Part model, mm, in its own coordinate system. A direction names the side the tool comes from. Coordinates: 2 decimals unless noted, no trailing zeros. Loops run counter-clockwise (first coordinate to the right, second up) from the corner with the lowest first, then second, coordinate; pieces in that order, holes last. Notation, with made-up numbers: (-17, -36) - (-8, -36) arc R27 ccw to (-8, -16) - close; hole circle Ø7 at (9, -15). An arc over 180 degrees is marked (long way). Answer as CSV lines item,"result".
from build123d import *

# Parameters (mm, degrees)
BOSS_EXTRUDE1_DEPTH = 6.4
SKETCH3_R           = 5
BOSS_EXTRUDE2_DEPTH = 30
CHAMFER1_SIZE       = 1


with BuildPart() as part:
    # Sketch1 → Boss-Extrude1 (new body)
    with BuildSketch(Plane.XY):
        Polygon((8, 4.618802154), (0, 9.237604307), (-8, 4.618802154), (-8, -4.618802154), (0, -9.237604307), (8, -4.618802154), align=None)
    extrude(amount=BOSS_EXTRUDE1_DEPTH)

    # Sketch3 → Boss-Extrude2 (add)
    with BuildSketch(Plane.XY.offset(6.4)):
        Circle(SKETCH3_R)
    extrude(amount=BOSS_EXTRUDE2_DEPTH)

    # Chamfer1
    chamfer1_edges = [part.edges().sort_by_distance(p)[0] for p in [
        (-5, 0, 36.4),
    ]]
    chamfer(chamfer1_edges, length=CHAMFER1_SIZE)


solid = part.part
Q1. Wall check: L1, parallel to Z at x = -4.5, y = -4; L2, parallel to X at y = -1.5, z = 8; L3, parallel to X at y = -0.75, z = 33.5. Give the ranges that are in metal, low to high.
Results:
L1,"z = 0 to 6.4"
L2,"x = -4.77 to 4.77"
L3,"x = -4.94 to 4.94"
Q2. Saw through at A-A (y = 0). Give the cut face in (x, z).
Results:
outline,"(-8, 0) - (8, 0) - (8, 6.4) - (5, 6.4) - (5, 35.4) - (4, 36.4) - (-4, 36.4) - (-5, 35.4) - (-5, 6.4) - (-8, 6.4) - close"
Q3. Saw through at D-D (y = -7.5). Give the cut face in (x, z), then the cut area to 3 significant figures.
Results:
outline,"(-3.01, 0) - (3.01, 0) - (3.01, 6.4) - (-3.01, 6.4) - close"
area,"38.5 mm^2"
Q4. Saw through at C-C (x = -5.5). Give the cut face in (y, z).
Results:
outline,"(-6.06, 0) - (6.06, 0) - (6.06, 6.4) - (-6.06, 6.4) - close"
Q5. Flat gauge pins, fed straight in: pin 1 (3 mm diameter, centred on x = -4.5, y = -4, fed in from -Z); pin 2 (6 mm diameter, centred on x = -4.5, z = 19.5, fed in from +Y); pin 3 (5 mm diameter, centred on y = 7, z = 9.5, fed in from +X); pin 4 (6 mm diameter, centred on y = -3, z = 16.5, fed in from -X). Where does each tip first touch, or does it go through?
Results:
pin 1,"stops at z = 0"
pin 2,"stops at y = 4.77"
pin 3,"stops at x = 2.18"
pin 4,"stops at x = -5"
Q6. Which spindle directions (+Z, -Z, +X, -X, +Y, -Y) get a long thin tool onto all of the face, cutting with end or side? Do faces 1 (the face through (0, 0, 0)), 2 (the face through (-1.08, -4.88, 20.7)). Say none if no direction does.
Results:
face 1,"-Z, +X, -X, +Y, -Y"
face 2,"+Z"
Q7. Saw through at B-B (z = 27.5). Give the cut face in (x, y).
Results:
outline,"circle Ø10 at (0, 0)"
